from build123d import *

# Parameters (mm, degrees)
SQUARE_TUBE_40_X_40_X_2_3_1_DEPTH = 1200


with BuildPart() as part:
    # Sketch11 → Square Tube 40 X 40 X 2.3(1) (new body)
    with BuildSketch(Plane.YZ):
        with BuildLine():
            Line((-15.4, -20), (15.4, -20))
            ThreePointArc((15.4, -20), (18.652691193, -18.652691193), (20, -15.4))
            Line((20, -15.4), (20, 15.4))
            ThreePointArc((20, 15.4), (18.652691193, 18.652691193), (15.4, 20))
            Line((15.4, 20), (-15.4, 20))
            ThreePointArc((-15.4, 20), (-18.652691193, 18.652691193), (-20, 15.4))
            Line((-20, 15.4), (-20, -15.4))
            ThreePointArc((-20, -15.4), (-18.652691193, -18.652691193), (-15.4, -20))
        make_face()
        with BuildLine():
            Line((-15.4, -17.7), (15.4, -17.7))
            ThreePointArc((15.4, -17.7), (17.026345597, -17.026345597), (17.7, -15.4))
            Line((17.7, -15.4), (17.7, 15.4))
            ThreePointArc((17.7, 15.4), (17.026345597, 17.026345597), (15.4, 17.7))
            Line((15.4, 17.7), (-15.4, 17.7))
            ThreePointArc((-15.4, 17.7), (-17.026345597, 17.026345597), (-17.7, 15.4))
            Line((-17.7, 15.4), (-17.7, -15.4))
            ThreePointArc((-17.7, -15.4), (-17.026345597, -17.026345597), (-15.4, -17.7))
        make_face(mode=Mode.SUBTRACT)
    extrude(amount=SQUARE_TUBE_40_X_40_X_2_3_1_DEPTH)


solid = part.part
Can you work these out from the model? Positions are in its coordinate system, mm. A direction names the side the tool comes from. Give positions to 0.01 mm unless a question says otherwise; leave off trailing zeros. Loops run counter-clockwise (first coordinate to the right, second up) from the corner with the lowest first, then second, coordinate; pieces in that order, holes last. Notation, with made-up numbers: (68.5, 10.25) - (92.5, 10.25) arc R23 cw to (92.5, 47.25) - close; hole circle Ø10 at (-16, 24.25). An arc over 180 degrees is marked (long way). One line per item, written item: value.
(1) If we section it at C-C, the plane x = 273: List the corners of the cut face in (y, z) for me.
Verdict:
outline: (-20, -15.4) arc R4.6 ccw to (-15.4, -20) - (15.4, -20) arc R4.6 ccw to (20, -15.4) - (20, 15.4) arc R4.6 ccw to (15.4, 20) - (-15.4, 20) arc R4.6 ccw to (-20, 15.4) - close; hole (-17.7, -15.4) arc R2.3 ccw to (-15.4, -17.7) - (15.4, -17.7) arc R2.3 ccw to (17.7, -15.4) - (17.7, 15.4) arc R2.3 ccw to (15.4, 17.7) - (-15.4, 17.7) arc R2.3 ccw to (-17.7, 15.4) - close
(2) I'm going to push a flat-ended pin straight in: pin 1 (2 mm diameter, centred on y = -15, z = -12, fed in from -X). Where does the tip first touch, or does it pass through?
Verdict:
pin 1: through
(3) If we mould it in two halves opening along Y, with no side actions, what happens to faces 1 (the face through (592, 0, 20)), 2 (the face through (592, 0, 17.7)), 3 (the face through (592, 20, 0))? For each: released by +Y, released by -Y, zero draft, split by the parting line, or undercut.
Verdict:
face 1: zero draft
face 2: undercut
face 3: released by +Y
(4) I need wall thicknesses on line 1 along Y through (x, z) = (957, 16); line 2 along Z through (x, y) = (415, -2). Which ranges of each line are inside material? Lowest first, please.
Verdict:
line 1: -19.96 to -17.62, 17.62 to 19.96
line 2: -20 to -17.7, 17.7 to 20
(5) If we section it at A-A, the plane z = -2: List the corners of the cut face in (x, y) for me, plus the area to 3 significant figures.
Verdict:
outline: (0, -20) - (1200, -20) - (1200, -17.7) - (0, -17.7) - close; (0, 17.7) - (1200, 17.7) - (1200, 20) - (0, 20) - close
area: 5,520 mm^2
(6) On a 3-axis mill with a long thin cutter (end or side, diameter ignored), from which of +Z, -Z, +X, -X, +Y, -Y can I reach the whole of each face in a straight line? I mean faces 4 (the face through (592, 0, -17.7)), 5 (the face through (592, 0, -20)). Say none if no direction works.
Verdict:
face 4: +X, -X
face 5: -Z, +X, -X, +Y, -Y
